```python
from build123d import *

# Parameters (mm, degrees)
EXTRUDE_962_DEPTH      = 1.25
EXTRUDE_962_DEPTH_BACK = 1.25
SKETCH_1_R             = 1.5


with BuildPart() as part:
    # 草图1 → Extrude 962 (new, two sides: drawn at the far end of the back side and taken through both)
    with BuildSketch(Plane.XY.offset(-EXTRUDE_962_DEPTH_BACK)):
        with BuildLine():
            Line((-10.833988703, -40.432996288), (-12.358609404, -46.122958205))
            ThreePointArc((-12.358609404, -46.122958205), (0, 47.75), (12.358609404, -46.122958205))
            Line((12.358609404, -46.122958205), (10.833988703, -40.432996288))
            ThreePointArc((10.833988703, -40.432996288), (13.272475808, -35.660239835), (18.269709097, -37.597527364))
            ThreePointArc((18.269709097, -37.597527364), (19.48154763, -38.613241212), (21.05227504, -38.43146483))
            ThreePointArc((21.05227504, -38.43146483), (0, 40.45), (-21.05227504, -38.43146483))
            ThreePointArc((-21.05227504, -38.43146483), (-19.48154763, -38.613241212), (-18.269709097, -37.597527364))
            ThreePointArc((-18.269709097, -37.597527364), (-13.272475808, -35.660239835), (-10.833988703, -40.432996288))
        make_face()
        with Locations((-14.866678993, -40.028388123)):
            Circle(SKETCH_1_R, mode=Mode.SUBTRACT)
        with Locations(Location((14.866678993, -40.028388123, 0), (0, 0, 180))):
            Circle(SKETCH_1_R, mode=Mode.SUBTRACT)
    extrude(amount=EXTRUDE_962_DEPTH + EXTRUDE_962_DEPTH_BACK)


solid = part.part
```
Read the model definition and answer for the solid it produces. Units are mm, in the model's axes. A direction names the side the tool comes from. Give positions to 0.01 mm unless a question says otherwise; leave off trailing zeros. Write each loop counter-clockwise with the first axis right and the second up, starting at its lowest first coordinate (ties: lowest second). Pieces come first, ordered by that corner, then holes. Notation, with made-up numbers: (-24, -29.5) -> (-10, -29.5) arc R22 cw to (-10, -19.5) -> close; hole circle Ø7 at (79, 25). An arc over 180 degrees is marked (long way). Answer in a Markdown table with one row per item.
1) Section D-D on x = 0 is taken. Give the vertices of the cut face in (y, z).
Results list:
| item | result |
|---|---|
| outline | (40.45, -1.25) -> (47.75, -1.25) -> (47.75, 1.25) -> (40.45, 1.25) -> close |
2) Each of these flat-tipped pins is pushed along its axis until it touches: pin 1 Ø1.5 at (y, z) = (-11, 1) entering from +X; pin 2 Ø1.5 at (x, z) = (35, -0.5) entering from +Y. Where does it stop, or does it pass through?
Results list:
| item | result |
|---|---|
| pin 1 | x = 46.64 |
| pin 2 | y = 33.27 |
3) A tool of negligible diameter and unlimited length cuts with its end or side. For faces 1 (the flat face through (14, 39, 1.25)), 2 (the cylindrical face through (-19.5, -38.62, -0.02)), 3 (the flat face through (11.607, -43.318, -0.018)), from which of +Z, -Z, +X, -X, +Y, -Y can it reach the whole face along a straight path? Write none if from no direction.
Results list:
| item | result |
|---|---|
| face 1 | +Z, +X, -X, +Y, -Y |
| face 2 | +Z, -Z |
| face 3 | +Z, -Z, -Y |
4) Section A-A on y = -17 is taken. Give the vertices of the cut face in (x, z).
Results list:
| item | result |
|---|---|
| outline | (-44.62, -1.25) -> (-39.42, -1.25) -> (-39.42, 1.25) -> (-44.62, 1.25) -> close; (39.42, -1.25) -> (44.62, -1.25) -> (44.62, 1.25) -> (39.42, 1.25) -> close |
5) Determine the mould class of faces 4 (the flat face through (14, 39, -1.25)), 5 (the cylindrical face through (-14.06, -38.764, -0.018)), 6 (the cylindrical face through (-1.92, 47.71, -0.02)), 7 (the cylindrical face through (13.2, -35.69, -0.02)) for opening direction X: released by +X, released by -X, zero draft, split by the parting line, or undercut.
Results list:
| item | result |
|---|---|
| face 4 | zero draft |
| face 5 | undercut |
| face 6 | split by the parting line |
| face 7 | undercut |
6) Section C-C on x = -37 is taken. Give the vertices of the cut face in (y, z).
Results list:
| item | result |
|---|---|
| outline | (-30.18, -1.25) -> (-22.2, -1.25) -> (-22.2, 1.25) -> (-30.18, 1.25) -> close; (18.6, -1.25) -> (30.18, -1.25) -> (30.18, 1.25) -> (18.6, 1.25) -> close |
7) Section B-B on z = 0.4 is taken. Give the vertices of the cut face in (x, y).
Results list:
| item | result |
|---|---|
| outline | (-21.05, -38.43) arc R42.25 cw (long way) to (21.05, -38.43) arc R2 cw to (18.27, -37.6) arc R4 ccw to (10.83, -40.43) -> (12.36, -46.12) arc R47.75 ccw (long way) to (-12.36, -46.12) -> (-10.83, -40.43) arc R4 ccw to (-18.27, -37.6) arc R2 cw to start; hole circle Ø3 at (-14.87, -40.03); hole circle Ø3 at (14.87, -40.03) |
8) Straight lines are drawn through the part: line 1 (Y direction, x = 32.5, z = -0.1); line 2 (X direction, y = 16, z = -0.7); line 3 (X direction, y = -8, z = -0.5). For each, find the intervals that lie inside material, in ascending order. Write a range as [from, to].
Results list:
| item | result |
|---|---|
| line 1 | [-34.98, -28.8], [25.2, 34.98] |
| line 2 | [-44.99, -38.32], [38.32, 44.99] |
| line 3 | [-47.08, -41.79], [41.79, 47.08] |
